Job drawing, mm, ordinate dimensions from the low corner. One solid piece. Coordinates: 2 decimals unless noted, no trailing zeros. Loops run counter-clockwise (first coordinate to the right, second up) from the corner with the lowest first, then second, coordinate; pieces in that order, holes last. Notation, with made-up numbers: M 13.25,-1 L 65.25,-1 A17 cw 65.25,31 Z; hole C -9.75,-8.5 d11. An arc over 180 degrees is marked long. Answer as a JSON object with one key per item and string values. Group by question number.
1. Saw through at C-C on z = 31. Write the cut outline in (x, y).
2. Saw through at B-B on y = 1. Write the cut outline in (x, z), then the cut area to 3 significant figures.
3. Drop flat-ended pins along their axis: pin 1 Ø4.5 at (x, z) = (25, 9.96) entering from +Y; pin 2 Ø5 at (x, z) = (21.5, 31.5) entering from -Y. Give the stop position or say it passes through.
4. Drill centre lines: L1, parallel to Z at x = 90, y = 1.8; L2, parallel to X at y = 1.85, z = 29.5; L3, parallel to X at y = 4.5, z = 29. Where is each one in solid material? Low to high.
5. Saw through at A-A on x = 25. Write the cut outline in (y, z).
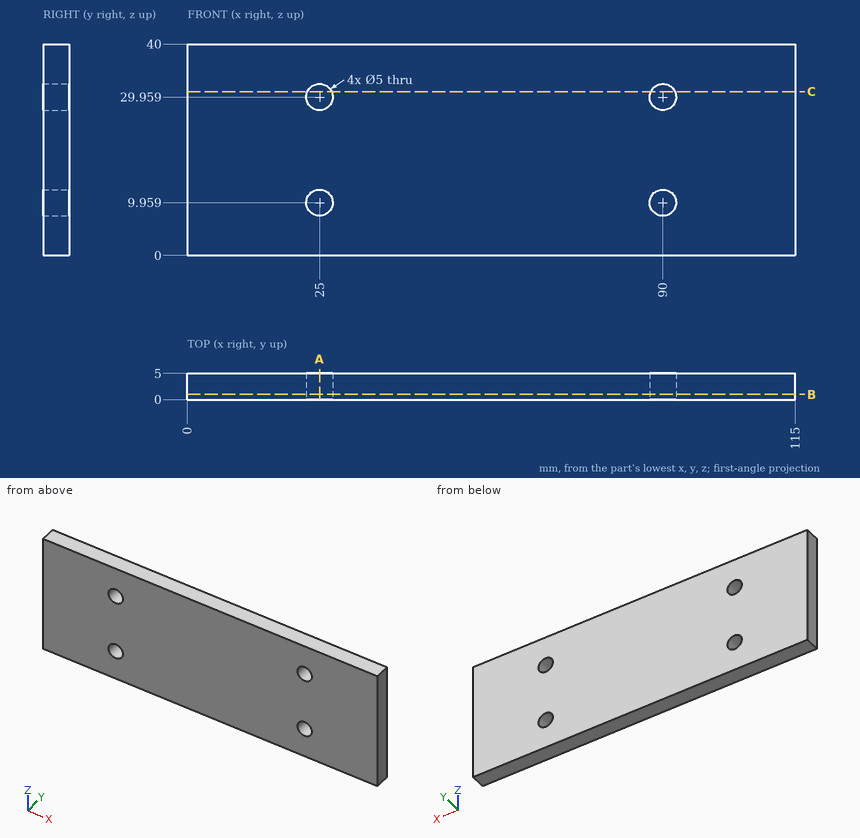
Outcome:
{
 "1": {"outline": "M 0,0 L 22.73,0 L 22.73,5 L 0,5 Z; M 27.27,0 L 87.73,0 L 87.73,5 L 27.27,5 Z; M 92.27,0 L 115,0 L 115,5 L 92.27,5 Z"},
 "2": {"outline": "M 0,0 L 115,0 L 115,40 L 0,40 Z; hole C 25,9.96 d5; hole C 25,29.96 d5; hole C 90,9.96 d5; hole C 90,29.96 d5", "area": "4,520 mm²"},
 "3": {"pin 1": "passes through", "pin 2": "stops at y = 0"},
 "4": {"L1": "z = 0 to 7.46, 12.46 to 27.46, 32.46 to 40", "L2": "x = 0 to 22.54, 27.46 to 87.54, 92.46 to 115", "L3": "x = 0 to 22.69, 27.31 to 87.69, 92.31 to 115"},
 "5": {"outline": "M 0,0 L 5,0 L 5,7.46 L 0,7.46 Z; M 0,12.46 L 5,12.46 L 5,27.46 L 0,27.46 Z; M 0,32.46 L 5,32.46 L 5,40 L 0,40 Z"}
}
